from build123d import *

# Parameters (mm, degrees)
SKETCH_1_W          = 206
SKETCH_1_H          = 146
EXTRUDE_1_DEPTH     = 1.5
SKETCH_2_R          = 35
CUT_EXTRUDE_1_DEPTH = 11.5


with BuildPart() as part:
    # 草图1 → 凸台-拉伸1 (new, symmetric)
    with BuildSketch(Plane.XY):
        Rectangle(SKETCH_1_W, SKETCH_1_H)
    extrude(amount=EXTRUDE_1_DEPTH, both=True)

    # 草图2 → 切除-拉伸1 (cut, symmetric)
    with BuildSketch(Plane.XY):
        Circle(SKETCH_2_R)
    extrude(amount=CUT_EXTRUDE_1_DEPTH, both=True, mode=Mode.SUBTRACT)


solid = part.part
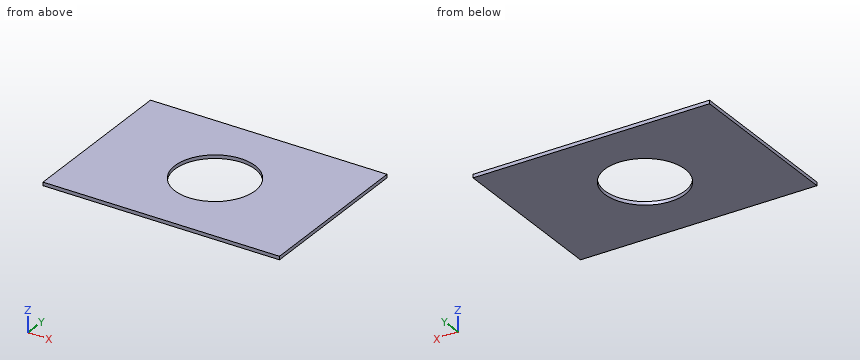
The listing builds one solid part. Answer for the finished solid, in the listing's coordinates (mm). Round coordinates to 2 decimals unless told otherwise and drop trailing zeros. Order: outer loops, then holes, each group sorted by start corner. A loop starts at its lowest first (then second) coordinate and runs counter-clockwise, first axis right, second up. Notation, with made-up numbers: (72.25, 44) - (98.25, 44) arc R21 ccw to (98.25, 48) - close; hole circle Ø6 at (65, -35.75). An arc over 180 degrees is marked (long way). Write item = value, one per line. Start each with the question number.
1) Section B-B, the plane y = -28 is taken. Write down the section's boundary in (x, z), plus the area to 3 significant figures.
2) Section C-C, the plane z = 0.9 is taken. Write down the section's boundary in (x, y).
3) Section A-A, the plane x = 0 is taken. Write down the section's boundary in (y, z).
4) Straight lines are drawn through the part: L1, parallel to Y at x = 0, z = -0.3; L2, parallel to X at y = 0.5, z = -0.4; L3, parallel to X at y = -2, z = 0.75. For each, find the intervals that lie inside material, in ascending order.
Results list:
q1.outline = (-103, -1.5) - (-21, -1.5) - (-21, 1.5) - (-103, 1.5) - close; (21, -1.5) - (103, -1.5) - (103, 1.5) - (21, 1.5) - close
q1.area = 492 mm^2
q2.outline = (-103, -73) - (103, -73) - (103, 73) - (-103, 73) - close; hole circle Ø70 at (0, 0)
q3.outline = (-73, -1.5) - (-35, -1.5) - (-35, 1.5) - (-73, 1.5) - close; (35, -1.5) - (73, -1.5) - (73, 1.5) - (35, 1.5) - close
q4.L1 = -73 to -35, 35 to 73
q4.L2 = -103 to -35, 35 to 103
q4.L3 = -103 to -34.94, 34.94 to 103
